Work out the finished part from the listing and answer in its coordinate system (mm). A direction names the side the tool comes from. Give positions to 0.01 mm unless a question says otherwise; leave off trailing zeros. Order: outer loops, then holes, each group sorted by start corner. A loop starts at its lowest first (then second) coordinate and runs counter-clockwise, first axis right, second up.
```python
from build123d import *

# Parameters (mm, degrees)
SKETCH_1_R          = 20
EXTRUDE_1_DEPTH     = 30.72
SKETCH_2_R          = 12.5
EXTRUDE_2_DEPTH     = 45
CUT_EXTRUDE_1_DEPTH = 25
CHAMFER_1_SIZE      = 1


with BuildPart() as part:
    # 草图1 → 凸台-拉伸1 (new body)
    with BuildSketch(Plane.XY):
        Circle(SKETCH_1_R)
    extrude(amount=EXTRUDE_1_DEPTH)

    # 草图2 → 凸台-拉伸2 (add)
    with BuildSketch(Plane.XY.offset(30.72)):
        with Locations(Location((0, 0, 0), (0, 0, 180))):
            Circle(SKETCH_2_R)
    extrude(amount=EXTRUDE_2_DEPTH)

    # 草图3 → 切除-拉伸1 (cut, symmetric)
    with BuildSketch(Plane(origin=(0, 0, 0), x_dir=(1, 0, 0), z_dir=(0, 1, 0))):
        Polygon((-20, 0), (20, 0), (-20, -10.72), align=None)
    extrude(amount=CUT_EXTRUDE_1_DEPTH, both=True, mode=Mode.SUBTRACT)

    # 倒角1
    chamfer_1_edges = [part.edges().sort_by_distance(p)[0] for p in [
        (-20, 0, 30.72),
        (12.5, 0, 75.72),
    ]]
    chamfer(chamfer_1_edges, length=CHAMFER_1_SIZE)


solid = part.part
```
1. The part is cut by section A-A (y = 0). Write down the section's boundary in (x, z), then the cut area to 3 significant figures.
Findings below:
outline: (-20, 10.72) - (20, 0) - (20, 29.72) - (19, 30.72) - (12.5, 30.72) - (12.5, 74.72) - (11.5, 75.72) - (-11.5, 75.72) - (-12.5, 74.72) - (-12.5, 30.72) - (-19, 30.72) - (-20, 29.72) - close
area: 2,140 mm2
2. Straight lines are drawn through the part: probe 1 along X at (y, z) = (0.5, 70); probe 2 along X at (y, z) = (7, 19) (3 decimals). For each, find the intervals that lie inside material, in ascending order.
Findings below:
probe 1: x = -12.49 to 12.49
probe 2: x = -18.735 to 18.735
3. The part is cut by section B-B (x = 0). Write down the section's boundary in (y, z), then the cut area to 3 significant figures.
Findings below:
outline: (-20, 5.36) - (20, 5.36) - (20, 29.72) - (19, 30.72) - (12.5, 30.72) - (12.5, 74.72) - (11.5, 75.72) - (-11.5, 75.72) - (-12.5, 74.72) - (-12.5, 30.72) - (-19, 30.72) - (-20, 29.72) - close
area: 2,140 mm2
4. The part is cut by section D-D (z = 19). Write down the section's boundary in (x, y).
Findings below:
outline: circle Ø40 at (0, 0)
5. Given P1, Ø4, axis at x = 10.5, z = 45.5, coming from the +Y side; P2, Ø8, axis at y = 11, z = 46.5, coming from the +X side; P3, Ø4, axis at y = -3, z = 29.5, coming from the -X side (3 decimals), each flat-ended and moving along its own axis, determine where each tip first touches the part or whether it passes through.
Findings below:
P1: stops at y = 9.17
P2: stops at x = 10.36
P3: stops at x = -19.975
6. Which of the six approach directions +Z, -Z, +X, -X, +Y, -Y give full straight-line access (tool end or side, diameter ignored) to faces 1 (the face through (19.076, 6.007, 17.954)), 2 (the face through (-11.923, -3.755, 52.412))?
Findings below:
face 1: +Z, -Z
face 2: +Z
7. The part is cut by section C-C (z = 47). Write down the section's boundary in (x, y), then the cut area to 3 significant figures.
Findings below:
outline: circle Ø25 at (0, 0)
area: 491 mm2
